Job drawing, mm, ordinate dimensions from the low corner. One solid piece. A direction names the side the tool comes from. Coordinates: 2 decimals unless noted, no trailing zeros. Loops run counter-clockwise (first coordinate to the right, second up) from the corner with the lowest first, then second, coordinate; pieces in that order, holes last. Notation, with made-up numbers: (-22.75, 7) - (-7.75, 7) arc R12 cw to (-7.75, 11) - close; hole circle Ø2 at (72.5, 31). An arc over 180 degrees is marked (long way). Use a Markdown table: item, result. Add a question column.
1. Band-saw the part on C-C, the plane y = 22. Give the cut face in (x, z), plus the area to 3 significant figures.
2. Pull direction X, two halves, no side cores. Call the marked faces 4, 5, 6 and 7: pulls with the +X half, pulls with the -X half, needs draft (parallel to the pull), parting line crosses it, or undercut.
3. Drop flat-ended pins along their axis: pin 1 (6 mm diameter, centred on y = 11.5, z = 2.5, fed in from -X); pin 2 (6 mm diameter, centred on x = 6.5, z = 7, fed in from +Y); pin 3 (10 mm diameter, centred on y = 30, z = 5, fed in from -X); pin 4 (8 mm diameter, centred on x = 9, z = 10, fed in from +Y). Give the stop position or say it passes through.
4. Band-saw the part on B-B, the plane z = 17.5. Give the cut face in (x, y).
5. 3-axis set-ups, long thin cutter, end or side, ignore diameter. For the marked faces 1, 2 and 3: which of +Z, -Z, +X, -X, +Y, -Y reach the whole face in a straight line?
6. Wall check: probe 1 along Z at (x, y) = (71, 1.65); probe 2 along X at (y, z) = (2, 11.25); probe 3 along Y at (x, z) = (40, 4.5). Give the ranges that are in metal, low to high. Write a range as [from, to].
7. Band-saw the part on A-A, the plane z = 10. Give the cut face in (x, y), plus the area to 3 significant figures.
8. Band-saw the part on D-D, the plane x = 71. Give the cut face in (y, z), plus the area to 3 significant figures.
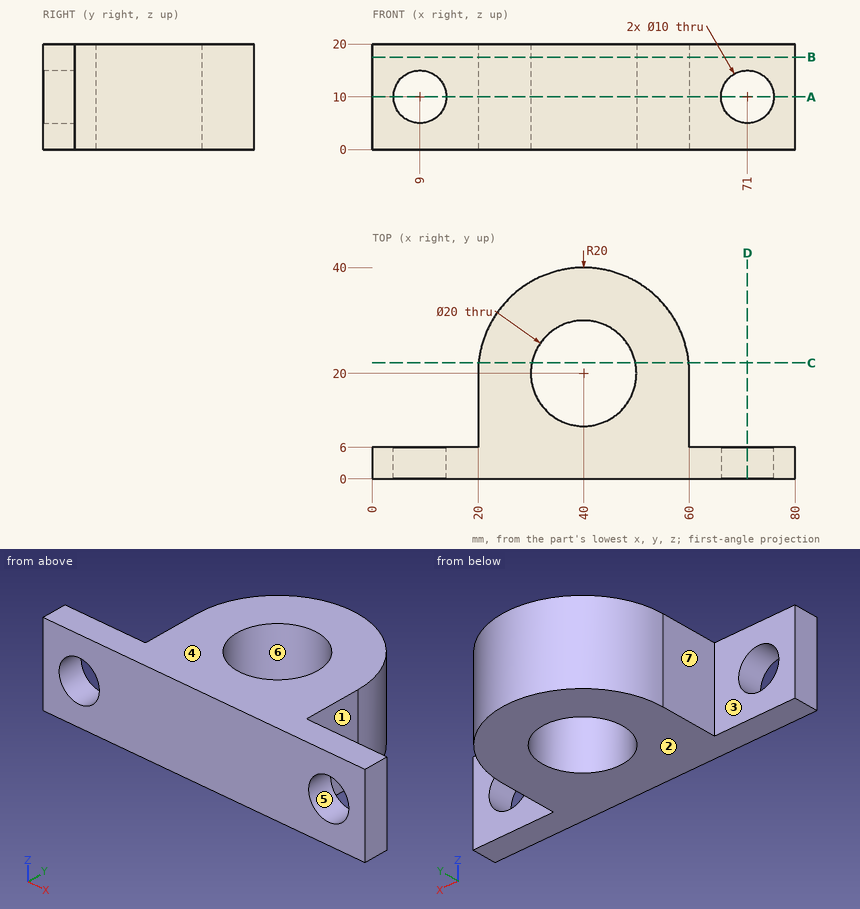
Geometry check:
| question | item | result |
|---|---|---|
| 1 | outline | (20.1, 0) - (30.2, 0) - (30.2, 20) - (20.1, 20) - close; (49.8, 0) - (59.9, 0) - (59.9, 20) - (49.8, 20) - close |
| 1 | area | 404 mm^2 |
| 2 | face 4 | needs draft |
| 2 | face 5 | undercut |
| 2 | face 6 | undercut |
| 2 | face 7 | pulls with the -X half |
| 3 | pin 1 | stops at x = 20 |
| 3 | pin 2 | stops at y = 6 |
| 3 | pin 3 | stops at x = 20.64 |
| 3 | pin 4 | passes through |
| 4 | outline | (0, 0) - (80, 0) - (80, 6) - (60, 6) - (60, 20) arc R20 ccw to (20, 20) - (20, 6) - (0, 6) - close; hole circle Ø20 at (40, 20) |
| 5 | face 1 | +Z, -Z, +X, +Y |
| 5 | face 2 | -Z, +X, -X, +Y, -Y |
| 5 | face 3 | +Z, -Z, -X, +Y |
| 6 | probe 1 | z = [0, 5], [15, 20] |
| 6 | probe 2 | x = [0, 4.16], [13.84, 66.16], [75.84, 80] |
| 6 | probe 3 | y = [0, 10], [30, 40] |
| 7 | outline | (0, 0) - (4, 0) - (4, 6) - (0, 6) - close; (14, 0) - (66, 0) - (66, 6) - (60, 6) - (60, 20) arc R20 ccw to (20, 20) - (20, 6) - (14, 6) - close; (76, 0) - (80, 0) - (80, 6) - (76, 6) - close; hole circle Ø20 at (40, 20) |
| 7 | area | 1,230 mm^2 |
| 8 | outline | (0, 0) - (6, 0) - (6, 5) - (0, 5) - close; (0, 15) - (6, 15) - (6, 20) - (0, 20) - close |
| 8 | area | 60.0 mm^2 |
